Source: CAD feature listing. Evaluate the final solid. Frame: model axes, mm. Face numbers are marked on the shaded views. A direction names the side the tool comes from. Round coordinates to 2 decimals unless told otherwise and drop trailing zeros. Order: outer loops, then holes, each group sorted by start corner. A loop starts at its lowest first (then second) coordinate and runs counter-clockwise, first axis right, second up.
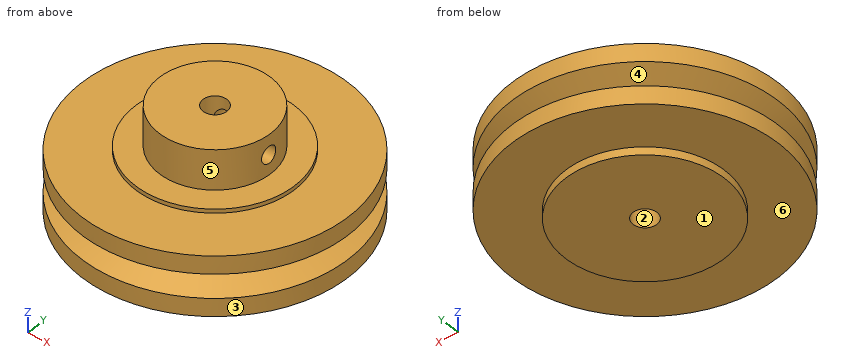
```python
from build123d import *

# Parameters (mm, degrees)
SKETCH1_R                       = 33.5
BOSS_EXTRUDE1_DEPTH             = 15
SKETCH4_R                       = 14
BOSS_EXTRUDE2_DEPTH             = 11
SKETCH3_R                       = 20
BOSS_EXTRUDE4_DEPTH             = 2
BOSS_EXTRUDE3_START             = 1
SKETCH2_R                       = 20
BOSS_EXTRUDE3_DEPTH             = 1
SKETCH5_R                       = 3
CUT_EXTRUDE3_DEPTH              = 56.031808984
M5_TAPPED_HOLE1_D               = 4.2
M5_TAPPED_HOLE1_DEPTH           = 13
M5_TAPPED_HOLE1_TIP             = 1.2618073
M5_TAPPED_HOLE1_ON_FACE_2_D     = 4.2
M5_TAPPED_HOLE1_ON_FACE_2_DEPTH = 13
M5_TAPPED_HOLE1_ON_FACE_2_TIP   = 1.2618073


with BuildPart() as part:
    # Sketch1 → Boss-Extrude1 (new body)
    with BuildSketch(Plane.XY):
        Circle(SKETCH1_R)
    extrude(amount=BOSS_EXTRUDE1_DEPTH)

    # Sketch4 → Boss-Extrude2 (add)
    with BuildSketch(Plane.XY.offset(15)):
        Circle(SKETCH4_R)
    extrude(amount=BOSS_EXTRUDE2_DEPTH)

    # Sketch3 → Boss-Extrude4 (add)
    with BuildSketch(Plane(origin=(0, 0, 0), x_dir=(-1, 0, 0), z_dir=(0, 0, -1))):
        Circle(SKETCH3_R)
    extrude(amount=BOSS_EXTRUDE4_DEPTH)

    # Sketch2 → Boss-Extrude3 (add)
    with BuildSketch(Plane.XY.offset(15).offset(BOSS_EXTRUDE3_START)):
        with Locations(Location((0, 0, 0), (0, 0, 180))):
            Circle(SKETCH2_R)
    extrude(amount=-BOSS_EXTRUDE3_DEPTH)

    # Sketch5 → Cut-Extrude3 (cut, through all)
    with BuildSketch(Plane.XY.offset(26)):
        Circle(SKETCH5_R)
    extrude(amount=-CUT_EXTRUDE3_DEPTH, mode=Mode.SUBTRACT)

    # Sketch7 → Cut-Revolve1 (revolve, cut)
    with BuildSketch(Plane(origin=(0, 0, 0), x_dir=(0, 0, -1), z_dir=(1, 0, 0)), mode=Mode.PRIVATE) as cut_revolve1_sk:
        Polygon((-8, 26.85), (-7, 26.85), (-4.5, 33.5), (-10.5, 33.5), align=None)
    revolve(cut_revolve1_sk.sketch.rotate(Axis((0, 0, 0), (0, 0, 1)), 90), axis=Axis((0, 0, 0), (0, 0, 1)), mode=Mode.SUBTRACT)

    # M5 Tapped Hole1
    with Locations(Plane(origin=(0, 14, 21), x_dir=(1, 0, 0), z_dir=(0, 1, 0))):
        with Locations((0, 0)):
            Hole(M5_TAPPED_HOLE1_D / 2, depth=M5_TAPPED_HOLE1_DEPTH)
            with Locations((0, 0, -(M5_TAPPED_HOLE1_DEPTH + M5_TAPPED_HOLE1_TIP / 2))):  # 118° drill point
                Cone(0, M5_TAPPED_HOLE1_D / 2, M5_TAPPED_HOLE1_TIP, mode=Mode.SUBTRACT)

    # M5 Tapped Hole1 on face 2
    with Locations(Plane(origin=(14, 0, 21), x_dir=(0, 0, 1), z_dir=(1, 0, 0))):
        with Locations((0, 0)):
            Hole(M5_TAPPED_HOLE1_ON_FACE_2_D / 2, depth=M5_TAPPED_HOLE1_ON_FACE_2_DEPTH)
            with Locations((0, 0, -(M5_TAPPED_HOLE1_ON_FACE_2_DEPTH + M5_TAPPED_HOLE1_ON_FACE_2_TIP / 2))):  # 118° drill point
                Cone(0, M5_TAPPED_HOLE1_ON_FACE_2_D / 2, M5_TAPPED_HOLE1_ON_FACE_2_TIP, mode=Mode.SUBTRACT)


solid = part.part
```
1. Line query: line 1 along Y through (x, z) = (0, 17.75); line 2 along Z through (x, y) = (0, 8); line 3 along Y through (x, z) = (0, 15.5). Output: solid intervals per line, ascending.
2. First-contact query: pin 1 (8 mm diameter, centred on x = -12, y = -16, fed in from +Z); pin 2 (1.5 mm diameter, centred on y = -12.5, z = 2, fed in from -X); pin 3 (4 mm diameter, centred on x = -10, z = 10, fed in from +Y). Flat tips, straight axial feed; report the tip coordinate or a pass-through.
3. Pull-direction query (Y, two-part tool) for the marked faces 1, 2 and 3; classes: released by +Y, released by -Y, zero draft, split by the parting line, or undercut.
4. Section D-D on z = 1.5. Return loops of the section in (x, y), plus the area to 3 significant figures.
5. Section C-C on z = 21. Return loops of the section in (x, y).
6. Access query for the marked faces 4, 5 and 6. Directions: +Z, -Z, +X, -X, +Y, -Y. A direction counts if a zero-diameter tool reaches every point of the face in a straight line with its end or side. Return the directions, or none.
7. Section A-A on y = 0. State how many separate pieces and enclosed holes the cut face has, plus the area to 3 significant figures.
Result:
1. line 1: y = -14 to -3, 3 to 14
1. line 2: z = -2 to 18.9, 23.1 to 26
1. line 3: y = -20 to -3, 3 to 20
2. pin 1: stops at z = 16
2. pin 2: stops at x = -31.37
2. pin 3: stops at y = 32.52
3. face 1: zero draft
3. face 2: undercut
3. face 3: split by the parting line
4. outline: circle Ø67 at (0, 0); hole circle Ø6 at (0, 0)
4. area: 3,500 mm2
5. outline: (-2.1, 2.14) - (-2.1, 13.84) arc R14 ccw (long way) to (13.84, -2.1) - (2.14, -2.1) arc R3 cw (long way) to start; (2.1, 2.14) arc R3 cw to (2.14, 2.1) - (13.84, 2.1) arc R14 ccw to (2.1, 13.84) - close
6. face 4: none
6. face 5: +Z
6. face 6: -Z
7. separate pieces: 3
7. enclosed holes: 0
7. area: 1,140 mm2
